```python
from build123d import *

# Parameters (mm, degrees)
SKETCH2_R           = 18
BOSS_EXTRUDE1_DEPTH = 50


with BuildPart() as part:
    # Sketch1 → Revolve1 (revolve)
    with BuildSketch(Plane.XY, mode=Mode.PRIVATE) as revolve1_sk:
        with BuildLine():
            Line((-24.494897428, 28), (-30, 28))
            Line((-30, 28), (-30, 8))
            Line((-30, 8), (-40, 8))
            Line((-40, 8), (-40, 0))
            Line((-40, 0), (0, 0))
            Line((0, 0), (0, 48))
            ThreePointArc((0, 48), (-15.811388301, 42.364916731), (-24.494897428, 28))
        make_face()
    revolve(revolve1_sk.sketch.rotate(Axis((0, 0, 0), (0, 1, 0)), 270), axis=Axis((0, 0, 0), (0, 1, 0)))

    # Sketch2 → Boss-Extrude1 (add)
    with BuildSketch(Plane(origin=(0, 0, 0), x_dir=(-1, 0, 0), z_dir=(0, -1, 0))):
        with Locations(Location((0, 0, 0), (0, 0, 90))):
            Circle(SKETCH2_R)
    extrude(amount=BOSS_EXTRUDE1_DEPTH)


solid = part.part
```
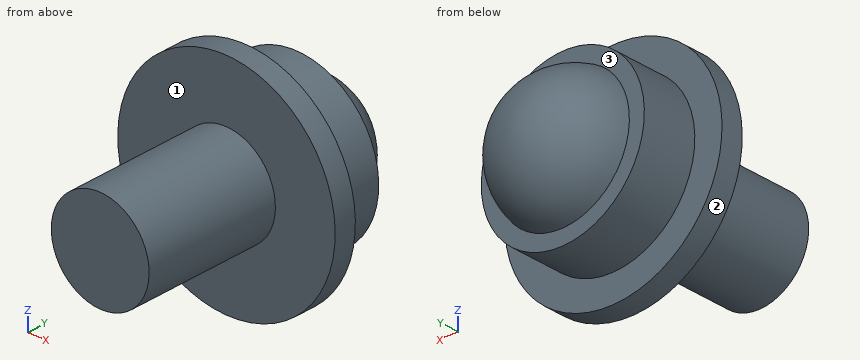
CAD build for the part. Positions are in the model's coordinates, mm. Face numbers are marked on the shaded views. A direction names the side the tool comes from. Coordinates: 2 decimals unless noted, no trailing zeros. Loops run counter-clockwise (first coordinate to the right, second up) from the corner with the lowest first, then second, coordinate; pieces in that order, holes last. Notation, with made-up numbers: (-22, 70) - (-2, 70) arc R7 ccw to (-2, 80) - close; hole circle Ø9 at (81.25, 32.5). An arc over 180 degrees is marked (long way). Return JSON: item names as keys, results as strings.
1. 3-axis set-ups, long thin cutter, end or side, ignore diameter. For the marked faces 1, 2 and 3: which of +Z, -Z, +X, -X, +Y, -Y reach the whole face in a straight line?
Result:
{"face 1": "-Y", "face 2": "+Y, -Y", "face 3": "+Y"}
2. Band-saw the part on B-B (x = 28). Give the cut face in (y, z).
Result:
{"outline": "(0, -28.57) - (8, -28.57) - (8, -10.77) - (28, -10.77) - (28, 10.77) - (8, 10.77) - (8, 28.57) - (0, 28.57) - close"}
3. Drop flat-ended pins along their axis: pin 1 (6 mm diameter, centred on y = 12.5, z = 29.5, fed in from +X); pin 2 (8 mm diameter, centred on x = -7.5, z = 30.5, fed in from +Y); pin 3 (6 mm diameter, centred on y = 7, z = 7.5, fed in from +X). Give the stop position or say it passes through.
Result:
{"pin 1": "stops at x = 14.06", "pin 2": "stops at y = 28", "pin 3": "stops at x = 39.75"}
4. Band-saw the part on D-D (x = 0). Give the cut face in (y, z).
Result:
{"outline": "(-50, -18) - (0, -18) - (0, -40) - (8, -40) - (8, -30) - (28, -30) - (28, -24.49) arc R25 ccw to (28, 24.49) - (28, 30) - (8, 30) - (8, 40) - (0, 40) - (0, 18) - (-50, 18) - close"}
5. Band-saw the part on C-C (y = 4). Give the cut face in (x, z).
Result:
{"outline": "circle Ø80 at (0, 0)"}
6. Probe L1, parallel to Z at x = 1, y = 12.5; L2, parallel to Z at x = 1, y = 1.5; L3, parallel to Y at x = -13.5, z = 33.5. List the from-to ranges inside material, lowest first. Write a range as from..to.
Result:
{"L1": "z = -29.98..29.98", "L2": "z = -39.99..39.99", "L3": "y = 0..8"}
7. Band-saw the part on A-A (z = 0). Give the cut face in (x, y), and give its area (3 significant figures).
Result:
{"outline": "(-40, 0) - (-18, 0) - (-18, -50) - (18, -50) - (18, 0) - (40, 0) - (40, 8) - (30, 8) - (30, 28) - (24.49, 28) arc R25 ccw to (-24.49, 28) - (-30, 28) - (-30, 8) - (-40, 8) - close", "area": "4,370 mm2"}
